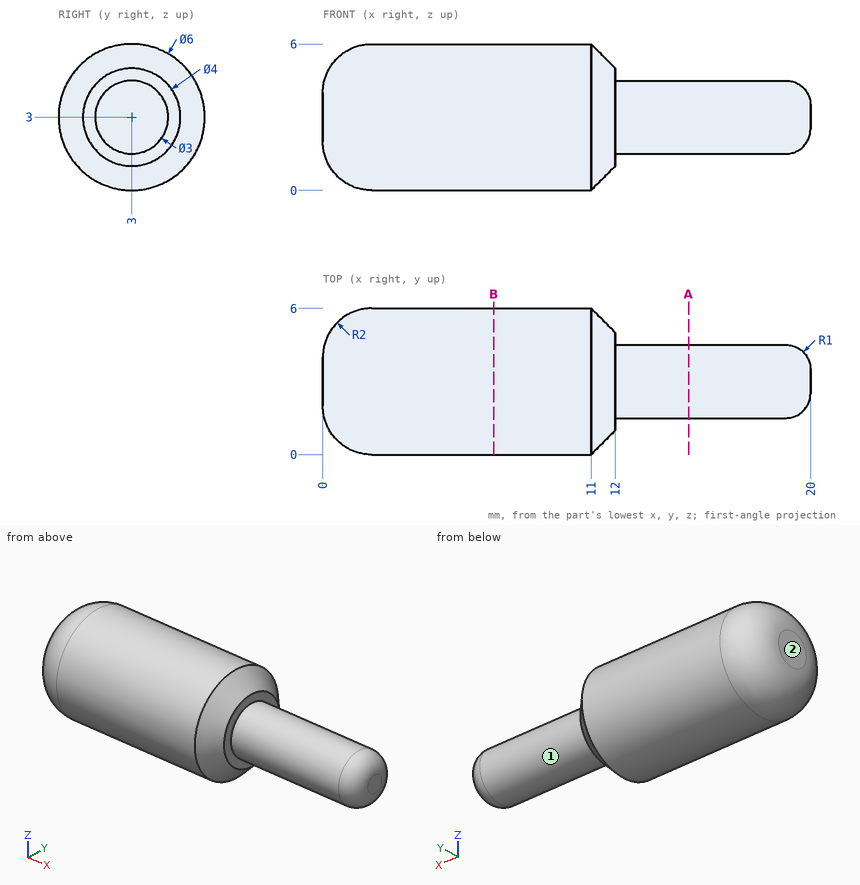
Could you check a few things on this drawing? It's one solid part, dimensions in mm from its lowest x, y, z. A direction names the side the tool comes from. Round coordinates to 2 decimals unless told otherwise and drop trailing zeros. Write each loop counter-clockwise with the first axis right and the second up, starting at its lowest first coordinate (ties: lowest second). Pieces come first, ordered by that corner, then holes. Notation, with made-up numbers: (82.5, 75.5) -> (108.5, 75.5) arc R16 cw to (108.5, 97.5) -> close; hole circle Ø6 at (-30, -30). An arc over 180 degrees is marked (long way). Use a Markdown table: item, result.
1. If we section it at A-A (x = 15): List the corners of the cut face in (y, z) for me.
Answer key:
| item | result |
|---|---|
| outline | circle Ø3 at (3, 3) |
2. If we section it at B-B (x = 7): List the corners of the cut face in (y, z) for me, then the cut area to 3 significant figures.
Answer key:
| item | result |
|---|---|
| outline | circle Ø6 at (3, 3) |
| area | 28.3 mm^2 |
3. Which directions (+Z, -Z, +X, -X, +Y, -Y) give clear straight access to the entire face, cutting with the end or side of a thin tool? Please do the marked faces 1 and 2.
Answer key:
| item | result |
|---|---|
| face 1 | +X |
| face 2 | +Z, -Z, -X, +Y, -Y |
4. For pin 1 Ø1 at (x, z) = (9.5, 2) entering from +Y; pin 2 Ø1.5 at (y, z) = (2.5, 1) entering from +X, each with a flat end and sliding along its axis, tell me the tip position at first contact or that it passes through.
Answer key:
| item | result |
|---|---|
| pin 1 | stops at y = 5.96 |
| pin 2 | stops at x = 19.58 |
5. Please list where these lines run through material, in increasing order: probe 1 along Y at (x, z) = (18, 2.95); probe 2 along X at (y, z) = (2.05, 3); probe 3 along X at (y, z) = (3.05, 1.65).
Answer key:
| item | result |
|---|---|
| probe 1 | y = 1.5 to 4.5 |
| probe 2 | x = 0 to 19.89 |
| probe 3 | x = 0.03 to 19.53 |
